Verification items for the finished model (mm, model axes). A direction names the side the tool comes from. Give positions to 0.01 mm unless a question says otherwise; leave off trailing zeros. Write each loop counter-clockwise with the first axis right and the second up, starting at its lowest first coordinate (ties: lowest second). Pieces come first, ordered by that corner, then holes. Notation, with made-up numbers: (41, 59.25) -> (64, 59.25) arc R9 cw to (64, 73.25) -> close; hole circle Ø8 at (-7, 19). An arc over 180 degrees is marked (long way). Use one line per item in the form item = value. Start each with the question number.
(1) Depth check by flat-ended pin: pin 1 Ø3 at (x, z) = (4.5, 35) entering from +Y; pin 2 Ø2 at (x, z) = (5, 27) entering from -Y; pin 3 Ø1.5 at (x, z) = (-1, 8.5) entering from +Y. Enter the tip coordinate at first touch or a pass-through.
(2) Scan lines: L1, parallel to Z at x = -3, y = 1.5; L2, parallel to Z at x = 5, y = -0.25; L3, parallel to Y at x = 5, z = 19 (3 decimals). Record each from-to range of solid material in increasing order.
(3) Section check C-C, the plane x = -3.5. Record the cut outline in (y, z).
(4) Section check A-A, the plane x = 0. Record the cut outline in (y, z), plus the area to 3 significant figures.
(5) Release check for a two-part mould opening along Z. For faces 4 (the face through (0, 0, 42)), 5 (the face through (5.08, 3.89, 27.21)), 6 (the face through (3, -1, 3)) record: pulls with the +Z half, pulls with the -Z half, needs draft (parallel to the pull), parting line crosses it, or undercut.
(6) Set-up check for faces 1 (the face through (0, 0, 0)), 2 (the face through (0.867, 3.905, 7.563)), 3 (the face through (2.9, -0.1, 2.5)): record each of +Z, -Z, +X, -X, +Y, -Y from which the full face is reachable in a straight line by a thin tool's end or side.
(7) Section check D-D, the plane z = 32.5. Record the cut outline in (x, y).
from build123d import *


with BuildPart() as part:
    # 草图1 → 旋转1 (revolve)
    with BuildSketch(Plane(origin=(0, 0, 0), x_dir=(1, 0, 0), z_dir=(0, 1, 0))):
        Polygon((0, 0), (-4, 0), (-4, -2), (-2.9, -2), (-2.9, -3), (-4, -3), (-4, -12), (-6.4, -12), (-6.4, -42), (0, -42), align=None)
    revolve(axis=Axis((0, 0, 0), (0, 0, 1)))


solid = part.part
Completed:
q1.pin_1 = 5.65
q1.pin_2 = -5
q1.pin_3 = 3.99
q2.L1 = 0 to 2, 3 to 42
q2.L2 = 12 to 42
q2.L3 = -3.995 to 3.995
q3.outline = (-5.36, 12) -> (-1.94, 12) -> (-1.94, 3) -> (1.94, 3) -> (1.94, 12) -> (5.36, 12) -> (5.36, 42) -> (-5.36, 42) -> close; (-1.94, 0) -> (1.94, 0) -> (1.94, 2) -> (-1.94, 2) -> close
q4.outline = (-6.4, 12) -> (-4, 12) -> (-4, 3) -> (-2.9, 3) -> (-2.9, 2) -> (-4, 2) -> (-4, 0) -> (4, 0) -> (4, 2) -> (2.9, 2) -> (2.9, 3) -> (4, 3) -> (4, 12) -> (6.4, 12) -> (6.4, 42) -> (-6.4, 42) -> close
q4.area = 478 mm²
q5.face_4 = pulls with the +Z half
q5.face_5 = needs draft
q5.face_6 = undercut
q6.face_1 = -Z, +X, -X, +Y, -Y
q6.face_2 = -Z
q6.face_3 = none
q7.outline = circle Ø12.8 at (0, 0)
